CAD build for the part. Positions are in the model's coordinates, mm. Face numbers are marked on the shaded views. Coordinates: 2 decimals unless noted, no trailing zeros. Order: outer loops, then holes, each group sorted by start corner. A loop starts at its lowest first (then second) coordinate and runs counter-clockwise, first axis right, second up. Notation, with made-up numbers: M 34,24.25 L 87,24.25 A27 ccw 87,53.25 Z; hole C 15.25,60.25 d2. An arc over 180 degrees is marked long. One line per item, written item: value.
from build123d import *

# Parameters (mm, degrees)
EXTRUDE_1_DEPTH                = 60
HOLE_WIZARD_M6_2_D             = 5
HOLE_WIZARD_M6_2_DEPTH         = 17
HOLE_WIZARD_M6_2_TIP           = 1.502151548
HOLE_WIZARD_M4_1_D             = 4.5
HOLE_WIZARD_M4_1_DEPTH         = 11.5
HOLE_WIZARD_M4_1_CBORE_D       = 8
HOLE_WIZARD_M4_1_CBORE_DEPTH   = 4.4
HOLE_WIZARD_M4_1_TIP           = 1.351936393
HOLE_WIZARD_M6_1_D             = 5
HOLE_WIZARD_M6_1_DEPTH         = 17
HOLE_WIZARD_M6_1_TIP           = 1.502151548
CHAMFER_1_SIZE                 = 3
SKETCH_9_W                     = 10
SKETCH_9_H                     = 44
CUT_EXTRUDE_1_DEPTH            = 109.166538369
CHAMFER_2_SIZE                 = 3
HOLE_WIZARD_M6_1_2_D           = 6.6
HOLE_WIZARD_M6_1_2_DEPTH       = 17
HOLE_WIZARD_M6_1_2_CBORE_D     = 11
HOLE_WIZARD_M6_1_2_CBORE_DEPTH = 6.4
HOLE_WIZARD_M6_1_2_TIP         = 1.982840043


with BuildPart() as part:
    # 草图2 → 凸台-拉伸1 (new body)
    with BuildSketch(Plane.XY):
        Polygon((0, 0), (0, -54), (72, -54), (72, -44), (10, -44), (10, 0), align=None)
    extrude(amount=EXTRUDE_1_DEPTH)

    # M6 螺纹孔2
    with Locations(Plane(origin=(0, 0, 0), x_dir=(-1, 0, 0), z_dir=(0, 0, -1))):
        with Locations((-60, -49)):
            Hole(HOLE_WIZARD_M6_2_D / 2, depth=HOLE_WIZARD_M6_2_DEPTH)
            with Locations((0, 0, -(HOLE_WIZARD_M6_2_DEPTH + HOLE_WIZARD_M6_2_TIP / 2))):  # 118° drill point
                Cone(0, HOLE_WIZARD_M6_2_D / 2, HOLE_WIZARD_M6_2_TIP, mode=Mode.SUBTRACT)

    # M4 六角凹头螺钉的柱形沉头孔1
    with Locations(Plane(origin=(0, -54, 0), x_dir=(-1, 0, 0), z_dir=(0, -1, 0))):
        with Locations((-40.299995099, -17), (-66.299995099, -17), (-66.299995099, -43), (-40.299995099, -43)):
            CounterBoreHole(HOLE_WIZARD_M4_1_D / 2, HOLE_WIZARD_M4_1_CBORE_D / 2, HOLE_WIZARD_M4_1_CBORE_DEPTH, depth=HOLE_WIZARD_M4_1_DEPTH)
            with Locations((0, 0, -(HOLE_WIZARD_M4_1_DEPTH + HOLE_WIZARD_M4_1_TIP / 2))):  # 118° drill point
                Cone(0, HOLE_WIZARD_M4_1_D / 2, HOLE_WIZARD_M4_1_TIP, mode=Mode.SUBTRACT)

    # Hole Wizard M6 _1
    with Locations(Plane(origin=(0, 0, 0), x_dir=(1, 0, 0), z_dir=(0, 1, 0))):
        with Locations((5, -15), (5, -45)):
            Hole(HOLE_WIZARD_M6_1_D / 2, depth=HOLE_WIZARD_M6_1_DEPTH)
            with Locations((0, 0, -(HOLE_WIZARD_M6_1_DEPTH + HOLE_WIZARD_M6_1_TIP / 2))):  # 118° drill point
                Cone(0, HOLE_WIZARD_M6_1_D / 2, HOLE_WIZARD_M6_1_TIP, mode=Mode.SUBTRACT)

    # 倒角1
    chamfer_1_edges = [part.edges().sort_by_distance(p)[0] for p in [
        (72, -49, 60),
        (5, 0, 60),
        (72, -49, 0),
        (5, 0, 0),
    ]]
    chamfer(chamfer_1_edges, length=CHAMFER_1_SIZE)

    # 草图9 → 切除-拉伸1 (cut, through all)
    with BuildSketch(Plane.XY.offset(60)):
        with Locations((5, -22)):
            Rectangle(SKETCH_9_W, SKETCH_9_H)
    extrude(amount=-CUT_EXTRUDE_1_DEPTH, mode=Mode.SUBTRACT)

    # 倒角2
    chamfer_2_edges = [part.edges().sort_by_distance(p)[0] for p in [
        (0, -49, 0),
        (0, -49, 60),
    ]]
    chamfer(chamfer_2_edges, length=CHAMFER_2_SIZE)

    # Hole Wizard M6 _1 2
    with Locations(Plane(origin=(0, -54, 0), x_dir=(-1, 0, 0), z_dir=(0, -1, 0))):
        with Locations((-5, -15), (-5, -45)):
            CounterBoreHole(HOLE_WIZARD_M6_1_2_D / 2, HOLE_WIZARD_M6_1_2_CBORE_D / 2, HOLE_WIZARD_M6_1_2_CBORE_DEPTH, depth=HOLE_WIZARD_M6_1_2_DEPTH)
            with Locations((0, 0, -(HOLE_WIZARD_M6_1_2_DEPTH + HOLE_WIZARD_M6_1_2_TIP / 2))):  # 118° drill point
                Cone(0, HOLE_WIZARD_M6_1_2_D / 2, HOLE_WIZARD_M6_1_2_TIP, mode=Mode.SUBTRACT)


solid = part.part
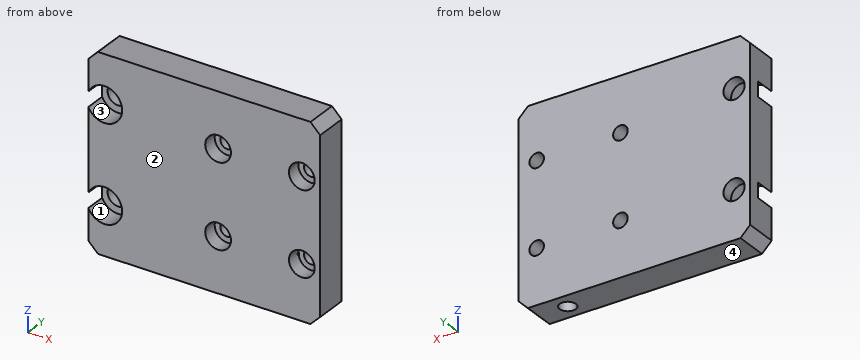
Q1. Slice it at B-B (x = 7). List the corners of the cut face in (y, z).
Recorded:
outline: M -54,0 L -44,0 L -44,12.38 L -47.6,12.38 L -47.6,9.88 L -54,9.88 Z; M -54,20.12 L -47.6,20.12 L -47.6,17.62 L -44,17.62 L -44,42.38 L -47.6,42.38 L -47.6,39.88 L -54,39.88 Z; M -54,50.12 L -47.6,50.12 L -47.6,47.62 L -44,47.62 L -44,60 L -54,60 Z
Q2. Pin check, flat tips, straight feed: pin 1 Ø7 at (x, z) = (40.3, 17) entering from -Y; pin 2 Ø5 at (x, z) = (66.3, 17) entering from +Y; pin 3 Ø5 at (x, z) = (3.5, 44) entering from -Y; pin 4 Ø6.5 at (x, z) = (5, 45) entering from +Y. Stop position of each tip, or through.
Recorded:
pin 1: stops at y = -49.6
pin 2: stops at y = -44
pin 3: stops at y = -47.6
pin 4: passes through
Q3. Drill centre lines: line 1 along Z through (x, y) = (5, -46.6); line 2 along Z through (x, y) = (5, -50); line 3 along X through (y, z) = (-45.25, 45). Where is each one in solid material? Low to high.
Recorded:
line 1: z = 0 to 11.7, 18.3 to 41.7, 48.3 to 60
line 2: z = 0 to 9.5, 20.5 to 39.5, 50.5 to 60
line 3: x = 0 to 1.7, 8.3 to 39.27, 41.33 to 65.27, 67.33 to 72
Q4. Mould opens along Z. For the marked faces 1, 2, 3 and 4 say: released by +Z, released by -Z, zero draft, split by the parting line, or undercut.
Recorded:
face 1: undercut
face 2: zero draft
face 3: undercut
face 4: released by -Z
Q5. Slice it at A-A (z = 4.5). List the corners of the cut face in (x, y), plus the area to 3 significant figures.
Recorded:
outline: M 0,-54 L 72,-54 L 72,-44 L 0,-44 Z; hole C 60,-49 d5
area: 700 mm^2
